```python
from build123d import *

# Parameters (mm, degrees)
SKETCH1_W           = 500
SKETCH1_H           = 320
SKETCH1_W_2         = 300
SKETCH1_H_2         = 260
BOSS_EXTRUDE1_DEPTH = 5
SKETCH2_W           = 303
SKETCH2_H           = 263
SKETCH2_W_2         = 300
SKETCH2_H_2         = 260
BOSS_EXTRUDE2_DEPTH = 170
SKETCH3_W           = 303
SKETCH3_H           = 263
SKETCH3_R           = 10
BOSS_EXTRUDE3_DEPTH = 1.5
FILLET2_R           = 10
FILLET3_R           = 11.5
SKETCH4_R           = 11.467682252
SKETCH4_R_2         = 9.967682252
BOSS_EXTRUDE4_DEPTH = 10
SKETCH5_R           = 7
CUT_EXTRUDE1_DEPTH  = 529.093031577
SKETCH6_R           = 10.66612067
BOSS_EXTRUDE5_DEPTH = 2


with BuildPart() as part:
    # Sketch1 → Boss-Extrude1 (new body)
    with BuildSketch(Plane.XY):
        with Locations((150, 130)):
            Rectangle(SKETCH1_W, SKETCH1_H)
        with Locations((150, 130)):
            Rectangle(SKETCH1_W_2, SKETCH1_H_2, mode=Mode.SUBTRACT)
    extrude(amount=BOSS_EXTRUDE1_DEPTH)

    # Sketch2 → Boss-Extrude2 (add)
    with BuildSketch(Plane.XY.offset(5)):
        with Locations((150, 130)):
            Rectangle(SKETCH2_W, SKETCH2_H)
        with Locations((150, 130)):
            Rectangle(SKETCH2_W_2, SKETCH2_H_2, mode=Mode.SUBTRACT)
    extrude(amount=BOSS_EXTRUDE2_DEPTH)

    # Sketch3 → Boss-Extrude3 (add)
    with BuildSketch(Plane.XY.offset(175)):
        with Locations((150, 130)):
            Rectangle(SKETCH3_W, SKETCH3_H)
        with Locations((140, 130)):
            Circle(SKETCH3_R, mode=Mode.SUBTRACT)
    extrude(amount=BOSS_EXTRUDE3_DEPTH)

    # Fillet2
    fillet2_edges = [part.edges().sort_by_distance(p)[0] for p in [
        (0, 260, 87.5),
        (0, 0, 87.5),
        (300, 0, 87.5),
        (300, 260, 87.5),
        (0, 130, 175),
        (150, 0, 175),
        (300, 130, 175),
        (150, 260, 175),
    ]]
    fillet(fillet2_edges, radius=FILLET2_R)

    # Fillet3
    fillet3_edges = [part.edges().sort_by_distance(p)[0] for p in [
        (-1.5, 261.5, 90.75),
        (-1.5, -1.5, 90.75),
        (301.5, -1.5, 90.75),
        (301.5, 261.5, 90.75),
        (301.5, 130, 176.5),
        (150, 261.5, 176.5),
        (-1.5, 130, 176.5),
        (150, -1.5, 176.5),
    ]]
    fillet(fillet3_edges, radius=FILLET3_R)

    # Sketch4 → Boss-Extrude4 (add)
    with BuildSketch(Plane.XY.offset(176.5)):
        with Locations(Location((140, 130, 0), (0, 0, 180))):
            Circle(SKETCH4_R)
        with Locations((140, 130)):
            Circle(SKETCH4_R_2, mode=Mode.SUBTRACT)
    extrude(amount=BOSS_EXTRUDE4_DEPTH)

    # Sketch5 → Cut-Extrude1 (cut, through all)
    with BuildSketch(Plane(origin=(0, 0, 0), x_dir=(-1, 0, 0), z_dir=(0, 0, -1))):
        with Locations((-20, -15)):
            Circle(SKETCH5_R)
        with Locations((-280, -15)):
            Circle(SKETCH5_R)
        with Locations((-20, 275)):
            Circle(SKETCH5_R)
        with Locations((-280, 275)):
            Circle(SKETCH5_R)
    extrude(amount=-CUT_EXTRUDE1_DEPTH, mode=Mode.SUBTRACT)

    # Sketch6 → Boss-Extrude5 (add)
    with BuildSketch(Plane(origin=(0, 0, 0), x_dir=(-1, 0, 0), z_dir=(0, 0, -1))):
        with Locations(Location((56.636018442, 245.08861857, 0), (0, 0, 180))):
            Circle(SKETCH6_R)
        with Locations(Location((56.636018442, 210.08861857, 0), (0, 0, 180))):
            Circle(SKETCH6_R)
        with Locations(Location((56.636018442, 175.08861857, 0), (0, 0, 180))):
            Circle(SKETCH6_R)
    extrude(amount=BOSS_EXTRUDE5_DEPTH)


solid = part.part
```
Part model, mm, in its own coordinate system. A direction names the side the tool comes from. Coordinates: 2 decimals unless noted, no trailing zeros. Order: outer loops, then holes, each group sorted by start corner. A loop starts at its lowest first (then second) coordinate and runs counter-clockwise, first axis right, second up. Notation, with made-up numbers: (35, 62) -> (68, 62) arc R35 ccw to (68, 96) -> close; hole circle Ø3 at (48.25, 10). An arc over 180 degrees is marked (long way). Put each result on its own line as item: value. Start each with the question number.
(1) Band-saw the part on C-C (y = 275). Give the cut face in (x, z).
(2) Pin check, flat tips, straight feed: pin 1 Ø10 at (x, y) = (241, 180) entering from -Z; pin 2 Ø12 at (x, y) = (-25, 30) entering from -Z; pin 3 Ø3 at (y, z) = (95, 115.5) entering from -X. Stop position of each tip, or through.
(3) Band-saw the part on D-D (x = 20). Give the cut face in (y, z).
(4) Probe line 1 along X through (y, z) = (275, 2); line 2 along X through (y, z) = (177, 136); line 3 along Y through (x, z) = (280, 2.4). List the from-to ranges inside material, lowest first. Write a range as [from, to].
(5) Which spindle directions (+Z, -Z, +X, -X, +Y, -Y) get a long thin tool onto all of the face, cutting with end or side? Do faces 1 (the face through (148, 261.5, 84)), 2 (the face through (-57, 175, -2)), 3 (the face through (148, -1.5, 84)), 4 (the face through (2.85, 131.68, 171.99)), 5 (the face through (145.38, 138.43, 175.74)). Say none if no direction does.
(6) Band-saw the part on B-B (z = 57). Give the cut face in (x, y).
(7) Mould opens along X. For faces 6 (the face through (-1.5, 128, 84)), 7 (the face through (147, 274, 0)), 8 (the face through (148, 0, 81)), 9 (the face through (-50.902, 201.095, -0.986)) say: pulls with the +X half, pulls with the -X half, needs draft (parallel to the pull), parting line crosses it, or undercut.
Determined:
1. outline: (-100, 0) -> (13, 0) -> (13, 5) -> (-100, 5) -> close; (27, 0) -> (273, 0) -> (273, 5) -> (27, 5) -> close; (287, 0) -> (400, 0) -> (400, 5) -> (287, 5) -> close
2. pin 1: stops at z = 175
2. pin 2: stops at z = 0
2. pin 3: stops at x = -1.5
3. outline: (-30, 0) -> (-22, 0) -> (-22, 5) -> (-30, 5) -> close; (-8, 0) -> (0, 0) -> (0, 165) arc R10 cw to (10, 175) -> (250, 175) arc R10 cw to (260, 165) -> (260, 0) -> (268, 0) -> (268, 5) -> (261.5, 5) -> (261.5, 165) arc R11.5 ccw to (250, 176.5) -> (10, 176.5) arc R11.5 ccw to (-1.5, 165) -> (-1.5, 5) -> (-8, 5) -> close; (282, 0) -> (290, 0) -> (290, 5) -> (282, 5) -> close
4. line 1: x = [-100, 13], [27, 273], [287, 400]
4. line 2: x = [-1.5, 0], [300, 301.5]
4. line 3: y = [-30, -22], [-8, 0], [260, 268], [282, 290]
5. face 1: +Z, +X, -X, +Y
5. face 2: -Z, +X, -X, +Y, -Y
5. face 3: +Z, +X, -X, -Y
5. face 4: -Z
5. face 5: +Z, -Z
6. outline: (-1.5, 10) arc R11.5 ccw to (10, -1.5) -> (290, -1.5) arc R11.5 ccw to (301.5, 10) -> (301.5, 250) arc R11.5 ccw to (290, 261.5) -> (10, 261.5) arc R11.5 ccw to (-1.5, 250) -> close; hole (0, 10) arc R10 ccw to (10, 0) -> (290, 0) arc R10 ccw to (300, 10) -> (300, 250) arc R10 ccw to (290, 260) -> (10, 260) arc R10 ccw to (0, 250) -> close
7. face 6: pulls with the -X half
7. face 7: needs draft
7. face 8: undercut
7. face 9: parting line crosses it
